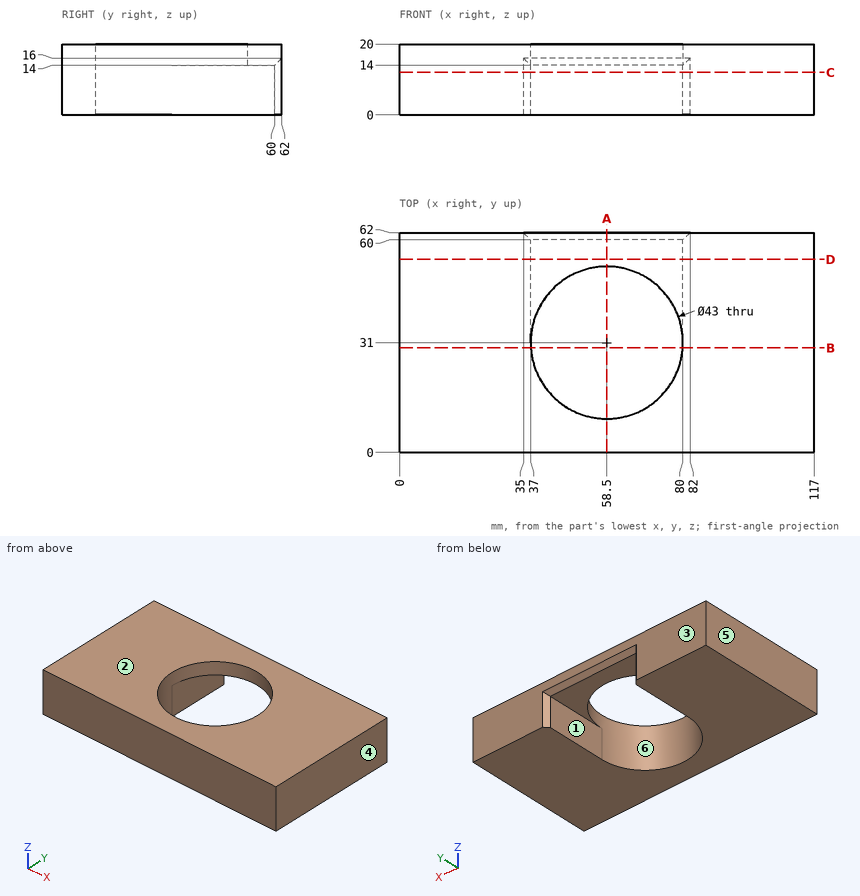
The figure shows three views and two pictorial views of one solid part (mm, origin at its lowest corner). Answer the questions. A direction names the side the tool comes from. Give positions to 0.01 mm unless a question says otherwise; leave off trailing zeros. Write each loop counter-clockwise with the first axis right and the second up, starting at its lowest first coordinate (ties: lowest second). Pieces come first, ordered by that corner, then holes. Notation, with made-up numbers: (65.25, 2) - (96.25, 2) arc R20 cw to (96.25, 17) - close; hole circle Ø6 at (35, -31.5). An arc over 180 degrees is marked (long way). Return JSON: item names as keys, results as strings.
Q1. For a pull along X with two mould halves and no side action, classify the marked faces 3, 4, 5 and 6 as released by +X, released by -X, zero draft, split by the parting line, or undercut.
Reply:
{"face 3": "zero draft", "face 4": "released by +X", "face 5": "released by -X", "face 6": "undercut"}
Q2. A cutting plane is placed at D-D, the plane y = 54.5. Determine the outline of the cut face in (x, z).
Reply:
{"outline": "(0, 0) - (37, 0) - (37, 14) - (80, 14) - (80, 0) - (117, 0) - (117, 20) - (0, 20) - close"}
Q3. A cutting plane is placed at A-A, the plane x = 58.5. Determine the outline of the cut face in (y, z).
Reply:
{"outline": "(0, 0) - (9.5, 0) - (9.5, 20) - (0, 20) - close; (52.5, 14) - (60, 14) - (62, 16) - (62, 20) - (52.5, 20) - close"}
Q4. Consider line 1 along X through (y, z) = (31, 11.25); line 2 along Y through (x, z) = (58.5, 11); line 3 along Y through (x, z) = (71.5, 17). Determine where each line is inside the solid, lowest interval first. Write a range as [from, to].
Reply:
{"line 1": "[0, 37], [80, 117]", "line 2": "[0, 9.5]", "line 3": "[0, 13.88], [48.12, 62]"}
Q5. A cutting plane is placed at C-C, the plane z = 12. Determine the outline of the cut face in (x, y).
Reply:
{"outline": "(0, 0) - (117, 0) - (117, 62) - (82, 62) - (80, 60) - (80, 31) arc R21.5 cw to (37, 31) - (37, 60) - (35, 62) - (0, 62) - close"}
Q6. A cutting plane is placed at B-B, the plane y = 29.5. Determine the outline of the cut face in (x, z), and give its area (3 significant figures).
Reply:
{"outline": "(0, 0) - (37.05, 0) - (37.05, 20) - (0, 20) - close; (79.95, 0) - (117, 0) - (117, 20) - (79.95, 20) - close", "area": "1,480 mm²"}
Q7. For the marked faces 1 and 2, determine the directions among +Z, -Z, +X, -X, +Y, -Y from which every point of the face is accessible in a straight line to the end or side of a thin tool.
Reply:
{"face 1": "-Z, +Y", "face 2": "+Z, +X, -X, +Y, -Y"}
Q8. Given P1, Ø2, axis at y = 40.5, z = 15.5, coming from the -X side; P2, Ø8.5, axis at x = 54.5, y = 45.5, coming from the -Z side, each flat-ended and moving along its own axis, determine where each tip first touches the part or whether it passes through.
Reply:
{"P1": "x = 0", "P2": "through"}
